```python
from build123d import *

# Parameters (mm, degrees)
SKETCH1_R           = 60
SKETCH1_R_2         = 30
BOSS_EXTRUDE1_DEPTH = 124
CUT_EXTRUDE1_START  = -31
SKETCH2_R           = 60
SKETCH2_R_2         = 55
CUT_EXTRUDE1_DEPTH  = 31
CHAMFER1_SIZE       = 2


with BuildPart() as part:
    # Sketch1 → Boss-Extrude1 (new body)
    with BuildSketch(Plane.XY):
        Circle(SKETCH1_R)
        Circle(SKETCH1_R_2, mode=Mode.SUBTRACT)
    extrude(amount=BOSS_EXTRUDE1_DEPTH)

    # Sketch2 → Cut-Extrude1 (cut)
    with BuildSketch(Plane.XY.offset(124).offset(CUT_EXTRUDE1_START)):
        Circle(SKETCH2_R)
        Circle(SKETCH2_R_2, mode=Mode.SUBTRACT)
    extrude(amount=CUT_EXTRUDE1_DEPTH, mode=Mode.SUBTRACT)

    # Chamfer1
    chamfer1_edges = [part.edges().sort_by_distance(p)[0] for p in [
        (-55, 0, 124),
        (-30, 0, 0),
        (-30, 0, 124),
    ]]
    chamfer(chamfer1_edges, length=CHAMFER1_SIZE)


solid = part.part
```
Can you work these out from the model? Positions are in its coordinate system, mm. A direction names the side the tool comes from. Round coordinates to 2 decimals unless told otherwise and drop trailing zeros. Loops run counter-clockwise (first coordinate to the right, second up) from the corner with the lowest first, then second, coordinate; pieces in that order, holes last.
Item 1: Will these pins go through, and if not, where does the flat tip stop? pin 1 Ø1.5 at (y, z) = (-47, 105.5) entering from -X; pin 2 Ø8 at (x, z) = (-8.5, 37.5) entering from -Y; pin 3 Ø10 at (y, z) = (-6, 106) entering from -X.
Item 2: Which directions (+Z, -Z, +X, -X, +Y, -Y) give clear straight access to the entire face, cutting with the end or side of a thin tool? Please do faces 5 (the flat face through (26, -49, 93)), 6 (the flat face through (23, -23, 124)).
Item 3: If we mould it in two halves opening along X, with no side actions, what happens to faces 1 (the cylindrical face through (-29.97, 1.32, 61.16)), 2 (the cylindrical face through (-11.923, -53.692, 107.297)), 3 (the conical face through (28.734, 9.049, 122.125)), 4 (the flat face through (26, -26, 0))? For each: +X half, -X half, draft (parallel to the pull), parting line (faces both ways), or undercut.
Item 4: Please list where these lines run through material, in increasing order: L1, parallel to Y at x = -0.5, z = 35; L2, parallel to Y at x = 0, z = 98; L3, parallel to Z at x = 12.5, y = -54.5.
Item 5: Suppose I cut it at A-A, the plane x = 0. Write out the boundary of the cut face in (y, z).
Item 6: Suppose I cut it at D-D, the plane z = 115. Write out the boundary of the cut face in (x, y).
Item 7: Suppose I cut it at C-C, the plane z = 56.5. Write out the boundary of the cut face in (x, y), then the cut area to 3 significant figures.
Reported:
1. pin 1: stops at x = -29.76
1. pin 2: stops at y = -59.83
1. pin 3: stops at x = -54.99
2. face 5: +Z
2. face 6: +Z, +X, -X, +Y, -Y
3. face 1: undercut
3. face 2: parting line
3. face 3: undercut
3. face 4: draft
4. L1: y = -60 to -30, 30 to 60
4. L2: y = -55 to -30, 30 to 55
4. L3: z = 0 to 93
5. outline: (-60, 0) - (-32, 0) - (-30, 2) - (-30, 122) - (-32, 124) - (-53, 124) - (-55, 122) - (-55, 93) - (-60, 93) - close; (30, 2) - (32, 0) - (60, 0) - (60, 93) - (55, 93) - (55, 122) - (53, 124) - (32, 124) - (30, 122) - close
6. outline: circle Ø110 at (0, 0); hole circle Ø60 at (0, 0)
7. outline: circle Ø120 at (0, 0); hole circle Ø60 at (0, 0)
7. area: 8,480 mm2
